Part model, mm, in its own coordinate system. A direction names the side the tool comes from. Round coordinates to 2 decimals unless told otherwise and drop trailing zeros. Write each loop counter-clockwise with the first axis right and the second up, starting at its lowest first coordinate (ties: lowest second). Pieces come first, ordered by that corner, then holes.
1) Pull direction Z, two halves, no side cores. Call faces 1 (the cylindrical face through (-61.08, -45.1, -49.56)), 2 (the cylindrical face through (54.45, -45.105, -82.494)), 3 (the flat face through (55, -52.5, -1)), 4 (the flat face through (-1, 55, 15)): +Z half, -Z half, draft (parallel to the pull), parting line (faces both ways), or undercut.
2) Flat gauge pins, fed straight in: pin 1 (7.5 mm diameter, centred on y = -43, z = 28, fed in from -X); pin 2 (25 mm diameter, centred on x = 57.5, z = -65, fed in from +Y); pin 3 (16.5 mm diameter, centred on y = 49.5, z = -23.5, fed in from -X); pin 4 (10 mm diameter, centred on y = -2, z = 52, fed in from -X). Where does each tip first touch, or does it go through?
3) Saw through at A-A on y = 0. Write the cut outline in (x, z).
4) Saw through at D-D on y = 64.5. Write the cut outline in (x, z).
5) Saw through at B-B on x = 55. Write the cut outline in (y, z).
6) Which spindle directions (+Z, -Z, +X, -X, +Y, -Y) get a long thin tool onto all of the face, cutting with end or side? Do faces 5 (the flat face through (-80, -47, -1)), 6 (the cylindrical face through (-2.44, 93.59, -22.4)), 7 (the flat face through (1, 38, 7.5)), 8 (the flat face through (30, -47, 1)). Say none if no direction does.
7) Saw through at C-C on z = -11. Write the cut outline in (x, y).
8) Drill centre lines: L1, parallel to X at y = -48, z = 57.5; L2, parallel to Y at x = 0, z = 20; L3, parallel to Z at x = -17, y = 83. Where is each one in solid material? Low to high.
```python
from build123d import *

# Parameters (mm, degrees)
SPLIT_SLEEVE_DEPTH                 = 95
SADDLE_BASE_PROFILE_W              = 50
SADDLE_BASE_PROFILE_H              = 15
SADDLE_BASE_DEPTH                  = 57.5
FOOT_TAB_DEPTH                     = 15
FOOT_TAB_MIRROR_RIGHT_COPY_1_DEPTH = 15
FOOT_MOUNTING_HOLES_4X_REACH       = 160.793
FOOT_HOLE_PROFILE_R                = 10
CLAMP_LUG_PROFILE_R                = 18.75
CLAMP_LUG_DEPTH                    = 15


with BuildPart() as part:
    # Split Sleeve Profile → Split Sleeve (new, symmetric)
    with BuildSketch(Plane(origin=(0, 0, 0), x_dir=(0, 0, -1), z_dir=(1, 0, 0))):
        with BuildLine():
            Line((-7.5, 44.370598373), (-7.5, 31.622776602))
            ThreePointArc((-7.5, 31.622776602), (0, -32.5), (7.5, 31.622776602))
            Line((7.5, 31.622776602), (7.5, 44.370598373))
            ThreePointArc((7.5, 44.370598373), (0, -45), (-7.5, 44.370598373))
        make_face()
    extrude(amount=SPLIT_SLEEVE_DEPTH, both=True)

    # Saddle Base Profile → Saddle Base (add, symmetric)
    with BuildSketch(Plane.XY):
        with Locations((-55, -45)):
            Rectangle(SADDLE_BASE_PROFILE_W, SADDLE_BASE_PROFILE_H)
        with Locations((55, -45)):
            Rectangle(SADDLE_BASE_PROFILE_W, SADDLE_BASE_PROFILE_H)
    extrude(amount=SADDLE_BASE_DEPTH, both=True)

    # Foot Tab Profile → Foot Tab (add)
    with BuildSketch(Plane.XZ.offset(52.5)):
        with BuildLine():
            Line((-80, 57.5), (-30, 57.5))
            ThreePointArc((-30, 57.5), (-55, 82.5), (-80, 57.5))
        make_face()
    foot_tab = extrude(amount=-FOOT_TAB_DEPTH)

    # Foot Tab Mirror Front: Foot Tab across plane
    add(foot_tab.mirror(Plane.XY))

    # Foot Tab Mirror Right: Foot Tab across plane
    add(foot_tab.mirror(Plane(origin=(0, 0, 0), x_dir=(0, 0, 1), z_dir=(1, 0, 0))))

    # Foot Tab Mirror Right copy 1 sketch → Foot Tab Mirror Right copy 1 (add)
    with BuildSketch(Plane(origin=(0, -52.5, 0), x_dir=(-1, 0, 0), z_dir=(0, -1, 0))):
        with BuildLine():
            Line((-80, 57.5), (-30, 57.5))
            ThreePointArc((-30, 57.5), (-55, 82.5), (-80, 57.5))
        make_face()
    extrude(amount=-FOOT_TAB_MIRROR_RIGHT_COPY_1_DEPTH)

    # Foot Hole Profile → Foot Mounting Holes 4x (cut, up to next)
    with BuildSketch(Plane.XZ.offset(52.5), mode=Mode.PRIVATE) as foot_mounting_holes_4x_sk1:
        with Locations(Location((-55, 57.5, 0), (0, 0, 270))):
            Circle(FOOT_HOLE_PROFILE_R)
    foot_mounting_holes_4x_tool1 = extrude(foot_mounting_holes_4x_sk1.sketch, amount=-FOOT_MOUNTING_HOLES_4X_REACH, mode=Mode.PRIVATE) & part.part
    # Foot Hole Profile → Foot Mounting Holes 4x (cut, up to next)
    with BuildSketch(Plane.XZ.offset(52.5), mode=Mode.PRIVATE) as foot_mounting_holes_4x_sk2:
        with Locations(Location((-55, -57.5, 0), (0, 0, 270))):
            Circle(FOOT_HOLE_PROFILE_R)
    foot_mounting_holes_4x_tool2 = extrude(foot_mounting_holes_4x_sk2.sketch, amount=-FOOT_MOUNTING_HOLES_4X_REACH, mode=Mode.PRIVATE) & part.part
    # Foot Hole Profile → Foot Mounting Holes 4x (cut, up to next)
    with BuildSketch(Plane.XZ.offset(52.5), mode=Mode.PRIVATE) as foot_mounting_holes_4x_sk3:
        with Locations(Location((55, -57.5, 0), (0, 0, 270))):
            Circle(FOOT_HOLE_PROFILE_R)
    foot_mounting_holes_4x_tool3 = extrude(foot_mounting_holes_4x_sk3.sketch, amount=-FOOT_MOUNTING_HOLES_4X_REACH, mode=Mode.PRIVATE) & part.part
    # Foot Hole Profile → Foot Mounting Holes 4x (cut, up to next)
    with BuildSketch(Plane.XZ.offset(52.5), mode=Mode.PRIVATE) as foot_mounting_holes_4x_sk4:
        with Locations(Location((55, 57.5, 0), (0, 0, 270))):
            Circle(FOOT_HOLE_PROFILE_R)
    foot_mounting_holes_4x_tool4 = extrude(foot_mounting_holes_4x_sk4.sketch, amount=-FOOT_MOUNTING_HOLES_4X_REACH, mode=Mode.PRIVATE) & part.part
    add(foot_mounting_holes_4x_tool1.solids().sort_by_distance((-55, -52.5, 57.5))[0], mode=Mode.SUBTRACT)
    add(foot_mounting_holes_4x_tool2.solids().sort_by_distance((-55, -52.5, -57.5))[0], mode=Mode.SUBTRACT)
    add(foot_mounting_holes_4x_tool3.solids().sort_by_distance((55, -52.5, -57.5))[0], mode=Mode.SUBTRACT)
    add(foot_mounting_holes_4x_tool4.solids().sort_by_distance((55, -52.5, 57.5))[0], mode=Mode.SUBTRACT)

    # Clamp Lug Profile → Clamp Lug (add)
    with BuildSketch(Plane.XY.offset(15)):
        with BuildLine():
            Line((-37.5, 75), (-37.5, 31.622776602))
            Line((-37.5, 31.622776602), (37.5, 31.622776602))
            Line((37.5, 31.622776602), (37.5, 75))
            ThreePointArc((37.5, 75), (0, 112.5), (-37.5, 75))
        make_face()
        with Locations((0, 75)):
            Circle(CLAMP_LUG_PROFILE_R, mode=Mode.SUBTRACT)
    clamp_lug = extrude(amount=CLAMP_LUG_DEPTH)

    # Clamp Lug Mirror: Clamp Lug across plane
    add(clamp_lug.mirror(Plane.XY))


solid = part.part
```
Completed:
1. face 1: undercut
1. face 2: -Z half
1. face 3: draft
1. face 4: undercut
2. pin 1: stops at x = -80
2. pin 2: stops at y = -37.5
2. pin 3: stops at x = -37.5
2. pin 4: passes through
3. outline: (-95, -45) - (95, -45) - (95, -32.5) - (-95, -32.5) - close; (-95, 32.5) - (95, 32.5) - (95, 45) - (-95, 45) - close
4. outline: (-37.5, -30) - (-15.53, -30) - (-15.53, -15) - (-37.5, -15) - close; (-37.5, 15) - (-15.53, 15) - (-15.53, 30) - (-37.5, 30) - close; (15.53, -30) - (37.5, -30) - (37.5, -15) - (15.53, -15) - close; (15.53, 15) - (37.5, 15) - (37.5, 30) - (15.53, 30) - close
5. outline: (-52.5, -82.5) - (-37.5, -82.5) - (-37.5, -67.5) - (-52.5, -67.5) - close; (-52.5, -47.5) - (-37.5, -47.5) - (-37.5, -24.87) arc R45 ccw to (44.37, -7.5) - (31.62, -7.5) arc R32.5 cw (long way) to (31.62, 7.5) - (44.37, 7.5) arc R45 ccw to (-37.5, 24.87) - (-37.5, 47.5) - (-52.5, 47.5) - close; (-52.5, 67.5) - (-37.5, 67.5) - (-37.5, 82.5) - (-52.5, 82.5) - close
6. face 5: -X, -Y
6. face 6: +Z, -Z
6. face 7: +X, -X, +Y
6. face 8: -Y
7. outline: (-95, -43.63) - (-80, -43.63) - (-80, -52.5) - (-30, -52.5) - (-30, -43.63) - (30, -43.63) - (30, -52.5) - (80, -52.5) - (80, -43.63) - (95, -43.63) - (95, -30.58) - (-95, -30.58) - close; (-95, 30.58) - (95, 30.58) - (95, 43.63) - (-95, 43.63) - close
8. L1: x = -80 to -65, -45 to -30, 30 to 45, 65 to 80
8. L2: y = -40.31 to -25.62, 25.62 to 56.25, 93.75 to 112.5
8. L3: z = -30 to -15, 15 to 30
